from build123d import *

# Parameters (mm, degrees)
HUB_PROFILE_R              = 15
HUB_30_DEPTH               = 30
BORE_PROFILE_R             = 6
BORE_12_DEPTH              = 60
ARM_DEPTH                  = 4
MOUNTING_PLATE_DEPTH       = 35
PLATE_LUG_DEPTH            = 10
MOUNTING_HOLES_PROFILE_R   = 5
MOUNTING_HOLES_2X_10_DEPTH = 87
SUPPORT_RIB_REACH          = 109.285
RIB_LINE_WALL_W            = 292.786132162
RIB_LINE_WALL_H            = 8


with BuildPart() as part:
    # Hub Profile → Hub Ø30 (new body)
    with BuildSketch(Plane(origin=(0, 0, 0), x_dir=(1, 0, 0), z_dir=(0, 1, 0))):
        with Locations(Location((0, 0, 0), (0, 0, 270))):
            Circle(HUB_PROFILE_R)
    extrude(amount=HUB_30_DEPTH)

    # Bore Profile → Bore Ø12 (cut)
    with BuildSketch(Plane(origin=(0, 30, 0), x_dir=(1, 0, 0), z_dir=(0, 1, 0))):
        with Locations(Location((0, 0, 0), (0, 0, 270))):
            Circle(BORE_PROFILE_R)
    extrude(amount=-BORE_12_DEPTH, mode=Mode.SUBTRACT)

    # Arm Profile → Arm (add, symmetric)
    with BuildSketch(Plane(origin=(0, 15, 0), x_dir=(1, 0, 0), z_dir=(0, 1, 0))):
        with BuildLine():
            Line((85, 0), (85, 37))
            Line((85, 37), (75, 37))
            Line((75, 37), (75, 23))
            ThreePointArc((75, 23), (72.656854249, 17.343145751), (67, 15))
            Line((67, 15), (0, 15))
            ThreePointArc((0, 15), (15, 0), (0, -15))
            Line((0, -15), (67, -15))
            ThreePointArc((67, -15), (72.656854249, -17.343145751), (75, -23))
            Line((75, -23), (75, -37))
            Line((75, -37), (85, -37))
            Line((85, -37), (85, 0))
        make_face()
    extrude(amount=ARM_DEPTH, both=True)

    # Mounting Plate Profile → Mounting Plate (add)
    with BuildSketch(Plane(origin=(0, 19, 0), x_dir=(1, 0, 0), z_dir=(0, 1, 0))):
        with BuildLine():
            Line((85, 0.780866297), (85, 25.780866297))
            Line((85, 25.780866297), (81, 25.780866297))
            ThreePointArc((81, 25.780866297), (74.301270189, 0.780866297), (81, -24.219133703))
            Line((81, -24.219133703), (85, -24.219133703))
            Line((85, -24.219133703), (85, 0.780866297))
        make_face()
    extrude(amount=MOUNTING_PLATE_DEPTH)

    # Plate Lug Profile → Plate Lug (add)
    with BuildSketch(Plane(origin=(85, 0, 0), x_dir=(0, 0, -1), z_dir=(1, 0, 0))):
        with BuildLine():
            Line((-37, 11), (-37, -27))
            ThreePointArc((-37, -27), (-31.142135624, -41.142135624), (-17, -47))
            Line((-17, -47), (17, -47))
            ThreePointArc((17, -47), (31.142135624, -41.142135624), (37, -27))
            Line((37, -27), (37, 11))
            Line((37, 11), (-37, 11))
        make_face()
    extrude(amount=-PLATE_LUG_DEPTH)

    # Mounting Holes Profile → Mounting Holes 2xØ10 (cut)
    with BuildSketch(Plane(origin=(85, 0, 0), x_dir=(0, 0, -1), z_dir=(1, 0, 0))):
        with Locations((22.5, -22)):
            Circle(MOUNTING_HOLES_PROFILE_R)
        with Locations((-22.5, -22)):
            Circle(MOUNTING_HOLES_PROFILE_R)
    extrude(amount=-MOUNTING_HOLES_2X_10_DEPTH, mode=Mode.SUBTRACT)

    # Rib Line wall → Support Rib (add, up to next)
    with BuildSketch(Plane(origin=(45, -23.5, 0), x_dir=(0.787228053529, -0.616661975264, 0), z_dir=(0.616661975264, 0.787228053529, 0)), mode=Mode.PRIVATE) as support_rib_sk1:
        Rectangle(RIB_LINE_WALL_W, RIB_LINE_WALL_H)
    support_rib_tool1 = extrude(support_rib_sk1.sketch, amount=SUPPORT_RIB_REACH, mode=Mode.PRIVATE) - part.part
    add(support_rib_tool1.solids().sort_by_distance((45, -23.5, 0))[0])


solid = part.part
The model under review builds one solid part; all positions refer to its coordinate system, in mm. A direction names the side the tool comes from. Round coordinates to 2 decimals unless told otherwise and drop trailing zeros. Loops run counter-clockwise (first coordinate to the right, second up) from the corner with the lowest first, then second, coordinate; pieces in that order, holes last. Notation, with made-up numbers: (13, -18.75) -> (44, -18.75) arc R35 ccw to (44, 18.25) -> close; hole circle Ø3 at (-27.5, 3). An arc over 180 degrees is marked (long way). One line per question, with ' | ' between items. Start each with the question number.
Item 1: Add section A-A, the plane y = 26. Write out the cut boundary in (x, z).
Item 2: Wall thickness on line 1 along X through (y, z) = (14.5, 0); line 2 along X through (y, z) = (-35, 20.5); line 3 along Y through (x, z) = (0.5, 12): over which ranges is each line inside the solid? List them lowest first. Write a range as [from, to].
Item 3: Add section C-C, the plane x = -4. Write out the cut boundary in (y, z).
Item 4: Add section B-B, the plane y = 14.5. Write out the cut boundary in (x, z), then the cut area to 3 significant figures.
Item 5: Machinability: for faces 1 (the face through (34, 15, -15)), 2 (the face through (0.2, 30, 6.5)), 3 (the face through (83, 36, 24.219)), 4 (the face through (83, 36, -25.781)), which of the approach directions +Z, -Z, +X, -X, +Y, -Y give a long, thin tool a straight path to every point of the face, cutting with its end or side? Answer none if there is none.
Item 6: Add section D-D, the plane y = -22. Write out the cut boundary in (x, z), then the cut area to 3 significant figures.
Item 7: Draft analysis for pull direction X (two halves, no side actions). For faces 5 (the face through (80.07, -40.986, 31.297)), 6 (the face through (74.303, 36.255, -1.147)), 7 (the face through (72.719, 15.056, -17.406)), state which applies: +X half, -X half, draft (parallel to the pull), parting line (faces both ways), or undercut.
Item 8: For pin 1 (17.5 mm diameter, centred on x = 51, y = -30, fed in from -Z); pin 2 (9 mm diameter, centred on x = 34, y = 14.5, fed in from +Z); pin 3 (2 mm diameter, centred on x = 71, z = -13.5, fed in from -Y), all flat-tipped, find the tip position at first contact; note any pin that passes through.
Return value:
1) outline: circle Ø30 at (0, 0); (81, -25.78) -> (85, -25.78) -> (85, 24.22) -> (81, 24.22) arc R50 ccw to start; hole circle Ø12 at (0, 0)
2) line 1: x = [-15, -6], [6, 85] | line 2: x = [75, 85] | line 3: y = [0, 30]
3) outline: (0, -14.46) -> (30, -14.46) -> (30, -4.47) -> (0, -4.47) -> close; (0, 4.47) -> (30, 4.47) -> (30, 14.46) -> (0, 14.46) -> close
4) outline: (0, -15) -> (67, -15) arc R8 cw to (75, -23) -> (75, -37) -> (85, -37) -> (85, 37) -> (75, 37) -> (75, 23) arc R8 cw to (67, 15) -> (0, 15) arc R15 ccw to start; hole circle Ø12 at (0, 0) | area: 3,260 mm2
5) face 1: -Z, -X, +Y, -Y | face 2: +Z, -Z, -X, +Y | face 3: +Z, +X, -X, +Y | face 4: -Z, +X, -X, +Y
6) outline: (43.09, -4) -> (75, -4) -> (75, -17.5) -> (85, -17.5) -> (85, 17.5) -> (75, 17.5) -> (75, 4) -> (43.09, 4) -> close; (75, -37) -> (85, -37) -> (85, -27.5) -> (75, -27.5) -> close; (75, 27.5) -> (85, 27.5) -> (85, 37) -> (75, 37) -> close | area: 795 mm2
7) face 5: draft | face 6: undercut | face 7: -X half
8) pin 1: stops at z = -4 | pin 2: stops at z = 15 | pin 3: stops at y = 11
